Geometry: final body of the model. Coordinates: model frame, mm. Give positions to 0.01 mm unless a question says otherwise; leave off trailing zeros. Order: outer loops, then holes, each group sorted by start corner. A loop starts at its lowest first (then second) coordinate and runs counter-clockwise, first axis right, second up. Notation, with made-up numbers: (0, 88) -> (9, 88) arc R31 cw to (9, 122) -> close; hole circle Ø5 at (78, 63.5). An arc over 180 degrees is marked (long way). One line per question, with ' | ' between items.
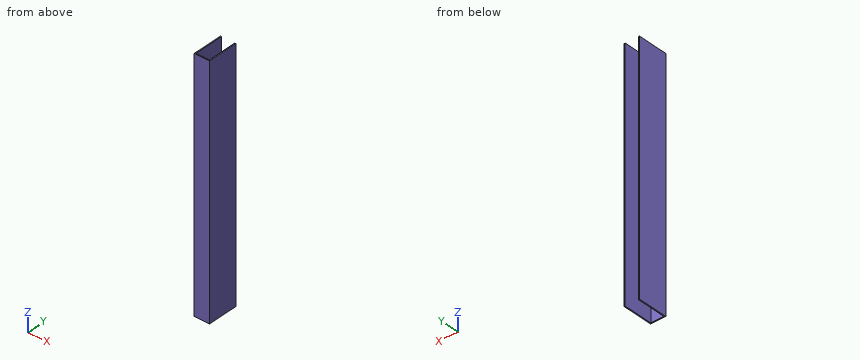
from build123d import *

# Parameters (mm, degrees)
SKETCH_1_W      = 30
SKETCH_1_H      = 60
EXTRUDE_1_DEPTH = 240
SHELL_1_T       = -2


with BuildPart() as part:
    # 草图1 → 凸台-拉伸1 (new, symmetric)
    with BuildSketch(Plane.XY):
        Rectangle(SKETCH_1_W, SKETCH_1_H)
    extrude(amount=EXTRUDE_1_DEPTH, both=True)

    # 抽壳1
    shell_1_openings = [part.faces().sort_by_distance(p)[0] for p in [
        (0, 0, 240),
        (0, 0, -240),
        (0, 30, 0),
    ]]
    offset(amount=SHELL_1_T, openings=shell_1_openings, kind=Kind.INTERSECTION)


solid = part.part
1) Contact query for a flat-ended pin moving along its axis: pin 1 Ø8 at (x, z) = (4, -40.5) entering from +Y. Output: stop coordinate, or through.
Check result:
pin 1: stops at y = -28
2) Section B-B on z = -62.5. Return loops of the section in (x, y).
Check result:
outline: (-15, -30) -> (15, -30) -> (15, 30) -> (13, 30) -> (13, -28) -> (-13, -28) -> (-13, 30) -> (-15, 30) -> close
3) Section C-C on x = -3.5. Return loops of the section in (y, z).
Check result:
outline: (-30, -240) -> (-28, -240) -> (-28, 240) -> (-30, 240) -> close
4) Material intervals for probe 1 along X at (y, z) = (9.5, 142); probe 2 along Y at (x, z) = (10, 164.5), sorted ascending. Write a range as from..to.
Check result:
probe 1: x = -15..-13, 13..15 | probe 2: y = -30..-28
5) Section A-A on y = -18.5. Return loops of the section in (x, z).
Check result:
outline: (-15, -240) -> (-13, -240) -> (-13, 240) -> (-15, 240) -> close; (13, -240) -> (15, -240) -> (15, 240) -> (13, 240) -> close
